from build123d import *

# Parameters (mm, degrees)
SKETCH1_W           = 40
SKETCH1_H           = 25
BOSS_EXTRUDE1_DEPTH = 8
SKETCH3_R           = 5
CUT_EXTRUDE1_DEPTH  = 48.843494856
SKETCH4_W           = 25
SKETCH4_H           = 1
CUT_EXTRUDE2_DEPTH  = 48.843494856
SKETCH7_W           = 18
SKETCH7_H           = 8
BOSS_EXTRUDE2_DEPTH = 20
CHAMFER2_SIZE       = 1
SKETCH8_R           = 4
CUT_EXTRUDE3_DEPTH  = 52.23475383
SKETCH9_R           = 2.5
CUT_EXTRUDE4_DEPTH  = 1
CUT_EXTRUDE5_START  = -1
SKETCH10_R          = 2.5
CUT_EXTRUDE5_DEPTH  = 1
SKETCH11_W          = 4
SKETCH11_H          = 4
BOSS_EXTRUDE3_DEPTH = 6
SKETCH12_R          = 1.5
CUT_EXTRUDE6_DEPTH  = 20
CHAMFER4_SIZE       = 1


with BuildPart() as part:
    # Sketch1 → Boss-Extrude1 (new body)
    with BuildSketch(Plane(origin=(0, 0, 0), x_dir=(1, 0, 0), z_dir=(0, 1, 0))):
        with Locations((20, -12.5)):
            Rectangle(SKETCH1_W, SKETCH1_H)
    extrude(amount=BOSS_EXTRUDE1_DEPTH)

    # Sketch3 → Cut-Extrude1 (cut, through all)
    with BuildSketch(Plane(origin=(0, 8, 0), x_dir=(1, 0, 0), z_dir=(0, 1, 0))):
        with Locations(Location((25, -12.5, 0), (0, 0, 270))):
            Circle(SKETCH3_R)
    extrude(amount=-CUT_EXTRUDE1_DEPTH, mode=Mode.SUBTRACT)

    # Sketch4 → Cut-Extrude2 (cut, through all)
    with BuildSketch(Plane(origin=(0, 8, 0), x_dir=(1, 0, 0), z_dir=(0, 1, 0))):
        with Locations((27.5, -12.5)):
            Rectangle(SKETCH4_W, SKETCH4_H)
    extrude(amount=-CUT_EXTRUDE2_DEPTH, mode=Mode.SUBTRACT)

    # Sketch7 → Boss-Extrude2 (add)
    with BuildSketch(Plane.XZ):
        with Locations((9, 4)):
            Rectangle(SKETCH7_W, SKETCH7_H)
        with Locations((9, 21)):
            Rectangle(SKETCH7_W, SKETCH7_H)
    extrude(amount=BOSS_EXTRUDE2_DEPTH)

    # Chamfer2
    chamfer2_edges = [part.edges().sort_by_distance(p)[0] for p in [
        (18, -20, 4),
        (18, -20, 21),
        (40, 4, 0),
        (40, 4, 25),
    ]]
    chamfer(chamfer2_edges, length=CHAMFER2_SIZE)

    # Sketch8 → Cut-Extrude3 (cut, through all)
    with BuildSketch(Plane(origin=(0, 0, 0), x_dir=(-1, 0, 0), z_dir=(0, 0, -1))):
        with Locations((-8.5, -12)):
            Circle(SKETCH8_R)
    extrude(amount=-CUT_EXTRUDE3_DEPTH, mode=Mode.SUBTRACT)

    # Sketch9 → Cut-Extrude4 (cut)
    with BuildSketch(Plane(origin=(0, 0, 0), x_dir=(-1, 0, 0), z_dir=(0, 0, -1))):
        with Locations((-29, 4)):
            Circle(SKETCH9_R)
        with Locations((-21, 4)):
            Circle(SKETCH9_R)
    extrude(amount=-CUT_EXTRUDE4_DEPTH, mode=Mode.SUBTRACT)

    # Sketch10 → Cut-Extrude5 (cut)
    with BuildSketch(Plane.XY.offset(25).offset(CUT_EXTRUDE5_START)):
        with Locations(Location((21, 4, 0), (0, 0, 180))):
            Circle(SKETCH10_R)
        with Locations(Location((29, 4, 0), (0, 0, 180))):
            Circle(SKETCH10_R)
    extrude(amount=CUT_EXTRUDE5_DEPTH, mode=Mode.SUBTRACT)

    # Sketch11 → Boss-Extrude3 (add)
    with BuildSketch(Plane.ZY):
        with Locations((19, -18)):
            Rectangle(SKETCH11_W, SKETCH11_H)
        with Locations((6, -18)):
            Rectangle(SKETCH11_W, SKETCH11_H)
    extrude(amount=BOSS_EXTRUDE3_DEPTH)

    # Sketch12 → Cut-Extrude6 (cut)
    with BuildSketch(Plane(origin=(0, 0, 4), x_dir=(-1, 0, 0), z_dir=(0, 0, -1))):
        with Locations((4, -18)):
            Circle(SKETCH12_R)
    extrude(amount=-CUT_EXTRUDE6_DEPTH, mode=Mode.SUBTRACT)

    # Chamfer4
    chamfer4_edges = [part.edges().sort_by_distance(p)[0] for p in [
        (0, -20, 2),
        (-6, -20, 6),
        (-6, -20, 19),
        (0, -20, 23),
    ]]
    chamfer(chamfer4_edges, length=CHAMFER4_SIZE)


solid = part.part
The model under review builds one solid part; all positions refer to its coordinate system, in mm. A direction names the side the tool comes from. Round coordinates to 2 decimals unless told otherwise and drop trailing zeros. Order: outer loops, then holes, each group sorted by start corner. A loop starts at its lowest first (then second) coordinate and runs counter-clockwise, first axis right, second up. Notation, with made-up numbers: (86, 77.5) -> (122, 77.5) arc R16 ccw to (122, 84.5) -> close; hole circle Ø5 at (14, 60). An arc over 180 degrees is marked (long way). Write item = value, one per line. Start each with the question number.
Item 1: For line 1 along Z through (x, y) = (34, 2); line 2 along Z through (x, y) = (1.5, -0.5); line 3 along Y through (x, z) = (-4, 7.1), list the stretches that pass through material, from the lowest coordinate up.
Item 2: Clearance check with flat-ended pins moving along their axes: pin 1 Ø8 at (y, z) = (3, 10) entering from -X; pin 2 Ø4 at (x, y) = (-4, -18) entering from +Z; pin 3 Ø3 at (x, y) = (21, 4) entering from +Z. State where each tip first meets the part, or that it passes through.
Item 3: Consider section B-B on x = 8.5. Write out the cut boundary in (y, z).
Item 4: Mouldability with a two-part tool opening along X and no side actions: class faces 4 (the face through (20, 0, 10)), 5 (the face through (11.7, -14.4, 20.9)), 6 (the face through (-6, -17, 19)) as released by +X, released by -X, zero draft, split by the parting line, or undercut.
Item 5: Consider section D-D on y = -1. Write out the cut boundary in (x, z).
Item 6: Consider section A-A on y = -18. Write out the cut boundary in (x, z), plus the area to 3 significant figures.
Item 7: Consider section C-C on z = 1.75. Write out the cut boundary in (x, y).
Item 8: For faces 1 (the face through (17, 4, 13)), 2 (the face through (21, 4, 24)), 3 (the face through (18, -9, 21)), list the 3-axis set-ups (+Z, -Z, +X, -X, +Y, -Y) from which the entire face can be reached by the end or side of a thin tool; tool diameter is ignored.
Conclusion:
q1.line_1 = 0 to 12, 13 to 25
q1.line_2 = 0 to 8, 17 to 25
q1.line_3 = -20 to -19.5, -16.5 to -16
q2.pin_1 = 0
q2.pin_2 = 21
q2.pin_3 = 24
q3.outline = (-20, 0) -> (-16, 0) -> (-16, 8) -> (-20, 8) -> close; (-20, 17) -> (-16, 17) -> (-16, 25) -> (-20, 25) -> close; (-8, 0) -> (8, 0) -> (8, 25) -> (-8, 25) -> (-8, 17) -> (0, 17) -> (0, 8) -> (-8, 8) -> close
q4.face_4 = zero draft
q4.face_5 = undercut
q4.face_6 = released by -X
q5.outline = (0, 0) -> (18, 0) -> (18, 8) -> (0, 8) -> close; (0, 17) -> (18, 17) -> (18, 25) -> (0, 25) -> close
q6.outline = (-6, 4) -> (-5.5, 4) -> (-5.5, 8) -> (-6, 8) -> close; (-6, 17) -> (-5.5, 17) -> (-5.5, 21) -> (-6, 21) -> close; (-2.5, 4) -> (0, 4) -> (0, 0) -> (18, 0) -> (18, 8) -> (-2.5, 8) -> close; (-2.5, 17) -> (18, 17) -> (18, 25) -> (0, 25) -> (0, 21) -> (-2.5, 21) -> close
q6.area = 312 mm2
q7.outline = (0, -19) -> (1, -20) -> (17, -20) -> (18, -19) -> (18, 0) -> (40, 0) -> (40, 8) -> (0, 8) -> close; hole circle Ø8 at (8.5, -12)
q8.face_1 = +X, +Y, -Y
q8.face_2 = +Z
q8.face_3 = +Z, -Z, +X, -Y
